Geometry check sheet. Reference: the model listing, model coordinates, mm. A direction names the side the tool comes from. Round coordinates to 2 decimals unless told otherwise and drop trailing zeros. Order: outer loops, then holes, each group sorted by start corner. A loop starts at its lowest first (then second) coordinate and runs counter-clockwise, first axis right, second up. Notation, with made-up numbers: (-14, 5) - (-8, 5) arc R17 ccw to (-8, 23) - close; hole circle Ø5 at (-11.75, -39). An arc over 180 degrees is marked (long way). Return JSON: item names as keys, results as strings. Group by question number.
Q1. Gauge pin test, flat ends, axial feed: pin 1 Ø3 at (x, z) = (22, -21) entering from -Y; pin 2 Ø16.5 at (x, y) = (-35, 4) entering from +Z; pin 3 Ø2 at (y, z) = (17.5, 23.5) entering from +X. Record the tip position at first contact, or that the pin passes through.
Q2. Sectioned sample at C-C, the plane y = 16.5. Record the cut outline in (x, z), then the cut area to 3 significant figures.
Q3. Material ranges on line 1 along Y through (x, z) = (57, 38); line 2 along X through (y, z) = (10, 0); line 3 along X through (y, z) = (24.5, -38), recorded low to high.
Q4. Sectioned sample at B-B, the plane z = 0. Record the cut outline in (x, y), then the cut area to 3 significant figures.
Q5. Sectioned sample at D-D, the plane x = 38. Record the cut outline in (y, z), then the cut area to 3 significant figures.
Q6. Draft check along X on faces 3 (the flat face through (-57, 3, 0)), 4 (the cylindrical face through (-4, 8, 20)), 5 (the cylindrical face through (66.523, 16.698, -33.154)). Enter one of: pulls with the +X half, pulls with the -X half, needs draft (parallel to the pull), parting line crosses it, or undercut.
Q7. Sectioned sample at A-A, the plane x = -40. Record the cut outline in (y, z).
Q8. Tool access check on faces 1 (the cylindrical face through (-3, 8, -21)), 2 (the flat face through (-40, 8, -27)). Record the directions out of +Z, -Z, +X, -X, +Y, -Y that give a thin tool (end or side, any length) a straight path to the whole face; none if there is none.
```python
from build123d import *

# Parameters (mm, degrees)
BASE_PLATE_SKETCH_W               = 114
BASE_PLATE_SKETCH_H               = 88
BASE_PLATE_114X88X15_DEPTH        = 15
FORK_EYE_A_SKETCH_R               = 24.1
FORK_EYE_A_48_2_DEPTH             = 22
FORK_START                        = -22
FORK_EYE_B_SKETCH_R               = 24.1
FORK_EYE_B_48_2_DEPTH             = 22
EYE_BORE_SKETCH_R                 = 12
EYE_BORE_24_DEPTH                 = 129.976044287
FORK_FILLET_R9_R                  = 9
FORK_GAP_PROFILE_SKETCH_R         = 10
FORK_GAP_AND_CLAMP_HOLE_CUT_DEPTH = 99.024588752
CLAMP_SLIT_2MM_DEPTH              = 119.033130942
CLAMP_SLIT_2MM_DEPTH_BACK         = 119.033130942
CLAMP_SLIT_SKETCH_W               = 32
CLAMP_SLIT_SKETCH_H               = 2


with BuildPart() as part:
    # Base Plate Sketch → Base Plate 114x88x15 (new body)
    with BuildSketch(Plane(origin=(0, 0, 0), x_dir=(1, 0, 0), z_dir=(0, 1, 0))):
        Rectangle(BASE_PLATE_SKETCH_W, BASE_PLATE_SKETCH_H)
    extrude(amount=BASE_PLATE_114X88X15_DEPTH)

    # Fork Eye A Sketch → Fork Eye A Ø48.2 (add)
    with BuildSketch(Plane.XY.offset(44)):
        with Locations((57, 24)):
            Circle(FORK_EYE_A_SKETCH_R)
    extrude(amount=-FORK_EYE_A_48_2_DEPTH)

    # Fork Eye B Sketch → Fork Eye B Ø48.2 (add)
    with BuildSketch(Plane(origin=(0, 0, -44), x_dir=(-1, 0, 0), z_dir=(0, 0, -1)).offset(FORK_START)):
        with Locations((-57, 24)):
            Circle(FORK_EYE_B_SKETCH_R)
    extrude(amount=FORK_EYE_B_48_2_DEPTH)

    # Eye Bore Sketch → Eye Bore Ø24 (cut, through all)
    with BuildSketch(Plane(origin=(0, 0, -44), x_dir=(-1, 0, 0), z_dir=(0, 0, -1))):
        with Locations((-57, 24)):
            Circle(EYE_BORE_SKETCH_R)
    extrude(amount=-EYE_BORE_24_DEPTH, mode=Mode.SUBTRACT)

    # Fork Fillet R9
    fork_fillet_r9_edges = [part.edges().sort_by_distance(p)[0] for p in [
        (34.643569158, 15, 33),
        (34.643569158, 15, -33),
    ]]
    fillet(fork_fillet_r9_edges, radius=FORK_FILLET_R9_R)

    # Fork Gap Profile Sketch → Fork Gap and Clamp Hole Cut (cut, through all)
    with BuildSketch(Plane(origin=(0, 15, 0), x_dir=(1, 0, 0), z_dir=(0, 1, 0))):
        with Locations(Location((-40, 0, 0), (0, 0, 270))):
            Circle(FORK_GAP_PROFILE_SKETCH_R)
        with BuildLine():
            Line((57, 22), (0, 22))
            ThreePointArc((0, 22), (-3.535533906, 20.535533906), (-5, 17))
            Line((-5, 17), (-5, -17))
            ThreePointArc((-5, -17), (-3.535533906, -20.535533906), (0, -22))
            Line((0, -22), (57, -22))
            Line((57, -22), (57, 22))
        make_face()
        with BuildLine():
            Line((-57, 44), (-7, 44))
            ThreePointArc((-7, 44), (-11.47918472, 32.186291501), (-23, 27))
            Line((-23, 27), (-57, 27))
            Line((-57, 27), (-57, 44))
        make_face()
        with BuildLine():
            Line((-57, -44), (-7, -44))
            ThreePointArc((-7, -44), (-11.47918472, -32.186291501), (-23, -27))
            Line((-23, -27), (-57, -27))
            Line((-57, -27), (-57, -44))
        make_face()
    extrude(amount=-FORK_GAP_AND_CLAMP_HOLE_CUT_DEPTH, mode=Mode.SUBTRACT)

    # Clamp Slit Sketch → Clamp Slit 2mm (cut, two sides: drawn at the far end of the back side and taken through both)
    with BuildSketch(Plane(origin=(0, 0, -27), x_dir=(-1, 0, 0), z_dir=(0, 0, -1)).offset(-CLAMP_SLIT_2MM_DEPTH_BACK)):
        with Locations((41, 6.5)):
            Rectangle(CLAMP_SLIT_SKETCH_W, CLAMP_SLIT_SKETCH_H)
    extrude(amount=CLAMP_SLIT_2MM_DEPTH + CLAMP_SLIT_2MM_DEPTH_BACK, mode=Mode.SUBTRACT)


solid = part.part
```
Reply:
{
 "1": {"pin 1": "y = 0", "pin 2": "z = 27", "pin 3": "x = 80.46"},
 "2": {"outline": "(28.87, -44) - (47.63, -44) - (47.63, -22) - (28.87, -22) - close; (28.87, 22) - (47.63, 22) - (47.63, 44) - (28.87, 44) - close; (66.37, -44) - (79.9, -44) - (79.9, -22) - (66.37, -22) - close; (66.37, 22) - (79.9, 22) - (79.9, 44) - (66.37, 44) - close", "area": "1,420 mm^2"},
 "3": {"line 1": "-0.1 to 12, 36 to 48.1", "line 2": "-57 to -50, -30 to -5", "line 3": "32.91 to 45.01, 68.99 to 81.09"},
 "4": {"outline": "(-57, 0) - (-50, 0) - (-50, 5.5) - (-57, 5.5) - close; (-57, 7.5) - (-50, 7.5) - (-50, 15) - (-57, 15) - close; (-30, 0) - (-5, 0) - (-5, 15) - (-30, 15) - (-30, 7.5) - (-25, 7.5) - (-25, 5.5) - (-30, 5.5) - close", "area": "456 mm^2"},
 "5": {"outline": "(0, -44) - (38.83, -44) - (38.83, -22) - (0, -22) - close; (0, 22) - (38.83, 22) - (38.83, 44) - (0, 44) - close", "area": "1,710 mm^2"},
 "6": {"face 3": "pulls with the -X half", "face 4": "pulls with the +X half", "face 5": "undercut"},
 "7": {"outline": "(0, -27) - (5.5, -27) - (5.5, -10) - (0, -10) - close; (0, 10) - (5.5, 10) - (5.5, 27) - (0, 27) - close; (7.5, -27) - (15, -27) - (15, -10) - (7.5, -10) - close; (7.5, 10) - (15, 10) - (15, 27) - (7.5, 27) - close"},
 "8": {"face 1": "+X, +Y, -Y", "face 2": "-Z, -X, +Y, -Y"}
}
